Work out the finished part from the listing and answer in its coordinate system (mm). Face numbers are marked on the shaded views. Coordinates: 2 decimals unless noted, no trailing zeros. Order: outer loops, then holes, each group sorted by start corner. A loop starts at its lowest first (then second) coordinate and runs counter-clockwise, first axis right, second up. Notation, with made-up numbers: M 85.5,-40 L 105.5,-40 A8 ccw 105.5,-33 Z; hole C -34,39 d6. An arc over 180 degrees is marked long. Answer in a Markdown table with one row per item. Add a question column.
Item 1: Consider line 1 (Z direction, x = 84.5, y = -32); line 2 (Y direction, x = -44, z = 39); line 3 (Y direction, x = -15, z = 36.5). Determine where each line is inside the solid, lowest interval first. Write a range as from..to.
Item 2: The part is cut by section D-D (y = 105). Write down the section's boundary in (x, z), then the cut area to 3 significant figures.
Item 3: The part is cut by section A-A (y = 0). State how many separate pieces and enclosed holes the cut face has, then the cut area to 3 significant figures.
Item 4: The mould has two halves that part along X. Classify the marked faces 1, 2 and 3: released by +X, released by -X, zero draft, split by the parting line, or undercut.
Item 5: The part is cut by section C-C (x = 108). Write down the section's boundary in (y, z).
Item 6: Flat-ended cylindrical pins translate along their axes: pin 1 Ø6 at (y, z) = (-83.5, 10.5) entering from -X; pin 2 Ø4 at (y, z) = (-77.5, 5.5) entering from +X; pin 3 Ø8 at (x, z) = (14.5, 22) entering from -Y. Find the tip coordinate at first contact, or state that the pin passes through.
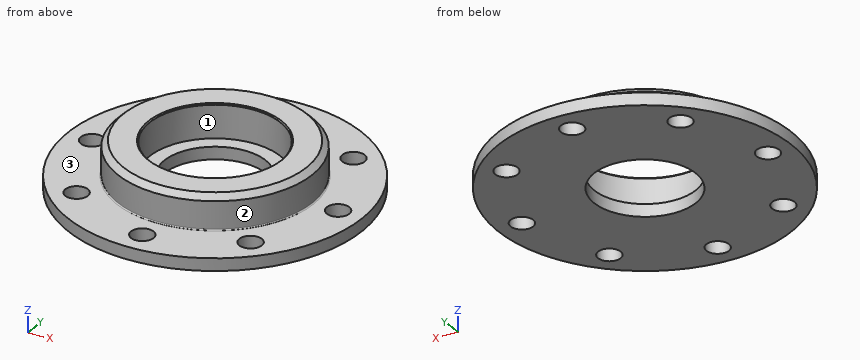
from build123d import *

# Parameters (mm, degrees)
SKETCH_1_R               = 130
EXTRUDE_1_DEPTH          = 11
SKETCH_2_R               = 86
SKETCH_2_R_2             = 58
EXTRUDE_2_DEPTH          = 30
FILLET_1_R               = 1
CHAMFER_1_SIZE           = 1
CHAMFER_2_SIZE           = 5
CUT_EXTRUDE_1_REACH      = 190.364
SKETCH_4_R               = 10
PATTERN_CIRCULAR_1_COUNT = 8
SKETCH_5_R               = 45
CUT_EXTRUDE_2_DEPTH      = 187.279360102


with BuildPart() as part:
    # 草图1 → 凸台-拉伸1 (new body)
    with BuildSketch(Plane.XY):
        Circle(SKETCH_1_R)
    extrude(amount=EXTRUDE_1_DEPTH)

    # 草图2 → 凸台-拉伸2 (add)
    with BuildSketch(Plane.XY.offset(11)):
        Circle(SKETCH_2_R)
        Circle(SKETCH_2_R_2, mode=Mode.SUBTRACT)
    extrude(amount=EXTRUDE_2_DEPTH)

    # 圆角1
    fillet_1_edges = [part.edges().sort_by_distance(p)[0] for p in [
        (-86, 0, 11),
    ]]
    fillet(fillet_1_edges, radius=FILLET_1_R)

    # 倒角1
    chamfer_1_edges = [part.edges().sort_by_distance(p)[0] for p in [
        (-58, 0, 41),
    ]]
    chamfer(chamfer_1_edges, length=CHAMFER_1_SIZE)

    # 倒角2
    chamfer_2_edges = [part.edges().sort_by_distance(p)[0] for p in [
        (-86, 0, 41),
    ]]
    chamfer(chamfer_2_edges, length=CHAMFER_2_SIZE)

    # 草图4 → 切除-拉伸1 (cut, up to next)
    with BuildSketch(Plane(origin=(0, 0, 0), x_dir=(-1, 0, 0), z_dir=(0, 0, -1)), mode=Mode.PRIVATE) as cut_extrude_1_sk1:
        with Locations((0, 108)):
            Circle(SKETCH_4_R)
    cut_extrude_1_tool1 = extrude(cut_extrude_1_sk1.sketch, amount=-CUT_EXTRUDE_1_REACH, mode=Mode.PRIVATE) & part.part
    cut_extrude_1 = cut_extrude_1_tool1.solids().sort_by_distance((0, 108, 0))[0]
    add(cut_extrude_1, mode=Mode.SUBTRACT)

    # 阵列(圆周)1: 切除-拉伸1 ×8 about axis
    pattern_circular_1_axis = Axis((0, 0, 0), (0, 0, 1))
    for i in range(1, PATTERN_CIRCULAR_1_COUNT):
        add(cut_extrude_1.rotate(pattern_circular_1_axis, i * 360 / PATTERN_CIRCULAR_1_COUNT), mode=Mode.SUBTRACT)

    # 草图5 → 切除-拉伸2 (cut, through all)
    with BuildSketch(Plane.XY.offset(11)):
        Circle(SKETCH_5_R)
    extrude(amount=-CUT_EXTRUDE_2_DEPTH, mode=Mode.SUBTRACT)


solid = part.part
Reply:
| question | item | result |
|---|---|---|
| 1 | line 1 | z = 0..11 |
| 1 | line 2 | y = -70.38..-37.79, 37.79..70.38 |
| 1 | line 3 | y = -84.17..-56.03, 56.03..84.17 |
| 2 | outline | M -76.65,0 L -9.54,0 L -9.54,11 L -76.65,11 Z; M 9.54,0 L 76.65,0 L 76.65,11 L 9.54,11 Z |
| 2 | area | 1,480 mm2 |
| 3 | separate pieces | 4 |
| 3 | enclosed holes | 0 |
| 3 | area | 3,080 mm2 |
| 4 | face 1 | undercut |
| 4 | face 2 | split by the parting line |
| 4 | face 3 | zero draft |
| 5 | outline | M -72.36,0 L -10,0 L -10,11 L -72.36,11 Z; M 10,0 L 72.36,0 L 72.36,11 L 10,11 Z |
| 6 | pin 1 | stops at x = -102.08 |
| 6 | pin 2 | stops at x = 105.83 |
| 6 | pin 3 | stops at y = -85.36 |
